Job drawing, mm, ordinate dimensions from the low corner. One solid piece. A direction names the side the tool comes from. Give positions to 0.01 mm unless a question says otherwise; leave off trailing zeros. Order: outer loops, then holes, each group sorted by start corner. A loop starts at its lowest first (then second) coordinate and runs counter-clockwise, first axis right, second up.
Item 1: Band-saw the part on B-B on z = 10. Give the cut face in (x, y), plus the area to 3 significant figures.
Item 2: Two-plate mould, pull along Z, no slides. Class the marked faces 4, 5 and 6: released by +Z, released by -Z, zero draft, split by the parting line, or undercut.
Item 3: Band-saw the part on C-C on y = 12.5. Give the cut face in (x, z), plus the area to 3 significant figures.
Item 4: Wall check: L1, parallel to Z at x = 63, y = 20.75; L2, parallel to Y at x = 66.5, z = 47; L3, parallel to Y at x = 35, z = 33. Give the ranges that are in metal, low to high.
Item 5: Band-saw the part on D-D on z = 18. Give the cut face in (x, y), plus the area to 3 significant figures.
Item 6: Band-saw the part on A-A on x = 7. Give the cut face in (y, z), plus the area to 3 significant figures.
Item 7: Flat gauge pins, fed straight in: P1, Ø9, axis at x = 63, z = 40, coming from the -Y side; P2, Ø8, axis at y = 5, z = 17.5, coming from the -X side; P3, Ø8, axis at y = 9, z = 27, coming from the -X side. Where does each tip first touch, or does it go through?
Item 8: Which spindle directions (+Z, -Z, +X, -X, +Y, -Y) get a long thin tool onto all of the face, cutting with end or side? Do the marked faces 1, 2 and 3. Say none if no direction does.
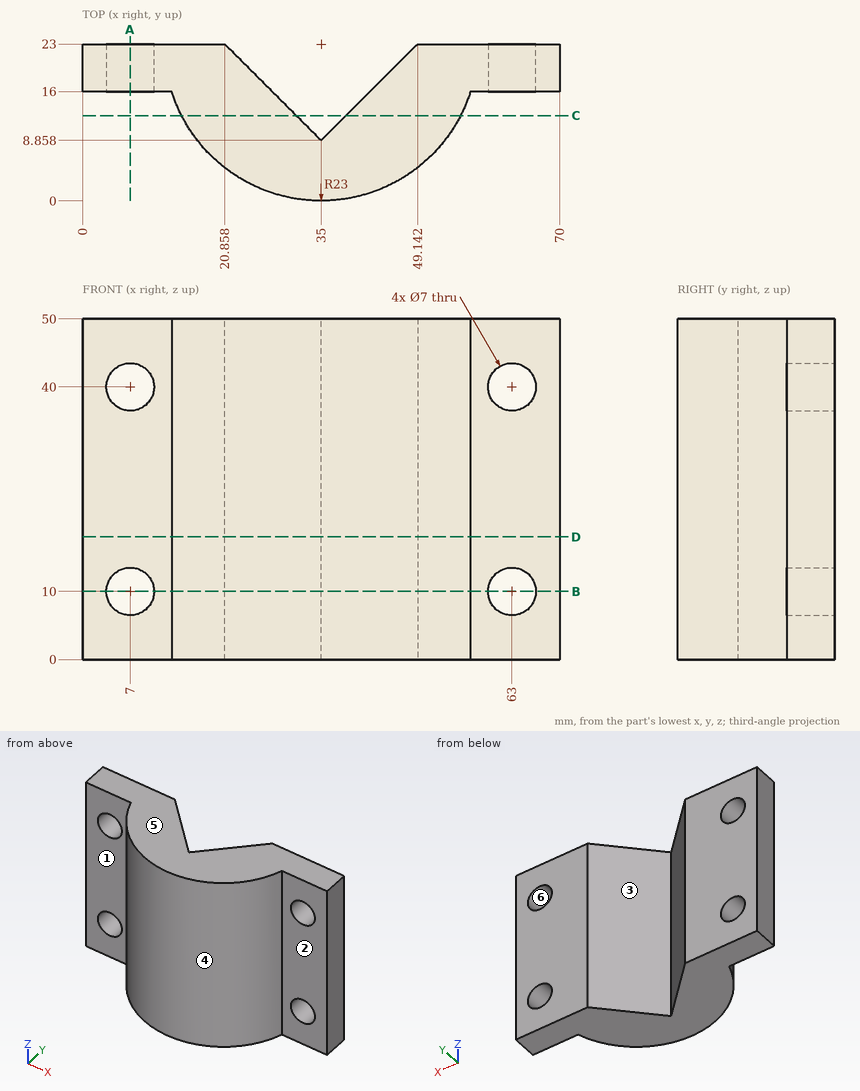
The answers:
1. outline: (0, 16) - (3.5, 16) - (3.5, 23) - (0, 23) - close; (10.5, 16) - (13.09, 16) arc R23 ccw to (56.91, 16) - (59.5, 16) - (59.5, 23) - (49.14, 23) - (35, 8.86) - (20.86, 23) - (10.5, 23) - close; (66.5, 16) - (70, 16) - (70, 23) - (66.5, 23) - close
1. area: 706 mm2
2. face 4: zero draft
2. face 5: released by +Z
2. face 6: undercut
3. outline: (14.54, 0) - (31.36, 0) - (31.36, 50) - (14.54, 50) - close; (38.64, 0) - (55.46, 0) - (55.46, 50) - (38.64, 50) - close
3. area: 1,680 mm2
4. L1: z = 0 to 6.5, 13.5 to 36.5, 43.5 to 50
4. L2: y = 16 to 23
4. L3: y = 0 to 8.86
5. outline: (0, 16) - (13.09, 16) arc R23 ccw to (56.91, 16) - (70, 16) - (70, 23) - (49.14, 23) - (35, 8.86) - (20.86, 23) - (0, 23) - close
5. area: 804 mm2
6. outline: (16, 0) - (23, 0) - (23, 6.5) - (16, 6.5) - close; (16, 13.5) - (23, 13.5) - (23, 36.5) - (16, 36.5) - close; (16, 43.5) - (23, 43.5) - (23, 50) - (16, 50) - close
6. area: 252 mm2
7. P1: stops at y = 16
7. P2: stops at x = 16.75
7. P3: stops at x = 14.29
8. face 1: +Z, -Z, -X, -Y
8. face 2: +Z, -Z, +X, -Y
8. face 3: +Z, -Z, +Y
